Design review of the part built by this model. Coordinates are the model's own, in mm. Face numbers are marked on the shaded views. A direction names the side the tool comes from. Give positions to 0.01 mm unless a question says otherwise; leave off trailing zeros. Loops run counter-clockwise (first coordinate to the right, second up) from the corner with the lowest first, then second, coordinate; pieces in that order, holes last. Notation, with made-up numbers: (53.25, 43) -> (86.25, 43) arc R16 cw to (86.25, 62) -> close; hole circle Ø10 at (-10.5, 67). An arc over 180 degrees is marked (long way). Answer in a Markdown table with one row per item. Add a question column.
(1) Consider section D-D on y = 14.25. Write out the cut boundary in (x, z).
(2) For the marked faces 4 and 5, list the 3-axis set-ups (+Z, -Z, +X, -X, +Y, -Y) from which the entire face can be reached by the end or side of a thin tool; tool diameter is ignored.
(3) Draft analysis for pull direction X (two halves, no side actions). For the marked faces 1, 2 and 3, state which applies: +X half, -X half, draft (parallel to the pull), parting line (faces both ways), or undercut.
(4) Consider section B-B on x = 0. Write out the cut boundary in (y, z), then the cut area to 3 significant figures.
(5) Consider section C-C on y = 7. Write out the cut boundary in (x, z), then the cut area to 3 significant figures.
(6) Consider section A-A on z = 0. Write out the cut boundary in (x, y).
(7) For pin 1 (6 mm diameter, centred on x = -0.5, y = 9, fed in from +Z); pin 2 (3.5 mm diameter, centred on x = 0, z = 0, fed in from -Y); pin 3 (1.5 mm diameter, centred on y = 6, z = -4, fed in from -X); pin 4 (8 mm diameter, centred on x = 5, y = 15, fed in from +Z), all flat-tipped, find the tip position at first contact; note any pin that passes through.
(8) For line 1 (X direction, y = 18, z = 0); line 2 (X direction, y = 12.75, z = 0); line 3 (Z direction, x = -1.75, y = 16), list the stretches that pass through material, from the lowest coordinate up.
from build123d import *

# Parameters (mm, degrees)
FILLET_1_R = 3
FILLET_2_R = 1


with BuildPart() as part:
    # 草图1 → 旋转1 (revolve)
    with BuildSketch(Plane.XY, mode=Mode.PRIVATE) as revolve_1_sk:
        Polygon((3, 25), (3, 0), (6, 0), (6, 13), (9, 13), (9, 25), align=None)
    revolve(revolve_1_sk.sketch.rotate(Axis((0, 0, 0), (0, 1, 0)), 90), axis=Axis((0, 0, 0), (0, 1, 0)))

    # 圆角1
    fillet_1_edges = [part.edges().sort_by_distance(p)[0] for p in [
        (0, 25, 9),
    ]]
    fillet(fillet_1_edges, radius=FILLET_1_R)

    # 圆角2
    fillet_2_edges = [part.edges().sort_by_distance(p)[0] for p in [
        (0, 0, 6),
    ]]
    fillet(fillet_2_edges, radius=FILLET_2_R)


solid = part.part
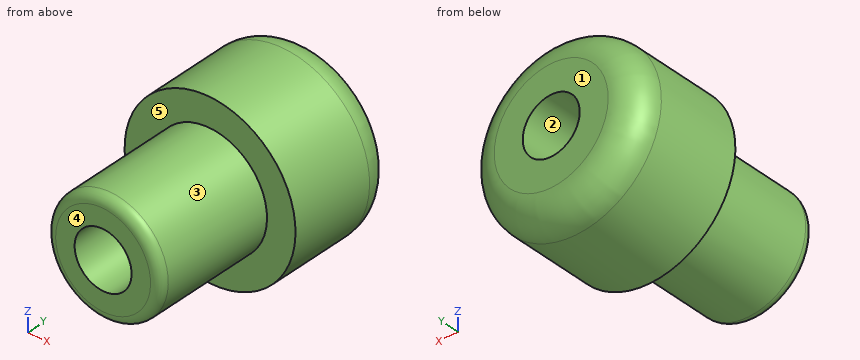
Values follow:
| question | item | result |
|---|---|---|
| 1 | outline | circle Ø18 at (0, 0); hole circle Ø6 at (0, 0) |
| 2 | face 4 | +Z, -Z, +X, -X, -Y |
| 2 | face 5 | -Y |
| 3 | face 1 | draft |
| 3 | face 2 | undercut |
| 3 | face 3 | parting line |
| 4 | outline | (0, -5) arc R1 ccw to (1, -6) -> (13, -6) -> (13, -9) -> (22, -9) arc R3 ccw to (25, -6) -> (25, -3) -> (0, -3) -> close; (0, 3) -> (25, 3) -> (25, 6) arc R3 ccw to (22, 9) -> (13, 9) -> (13, 6) -> (1, 6) arc R1 ccw to (0, 5) -> close |
| 4 | area | 218 mm2 |
| 5 | outline | circle Ø12 at (0, 0); hole circle Ø6 at (0, 0) |
| 5 | area | 84.8 mm2 |
| 6 | outline | (-9, 13) -> (-6, 13) -> (-6, 1) arc R1 ccw to (-5, 0) -> (-3, 0) -> (-3, 25) -> (-6, 25) arc R3 ccw to (-9, 22) -> close; (3, 0) -> (5, 0) arc R1 ccw to (6, 1) -> (6, 13) -> (9, 13) -> (9, 22) arc R3 ccw to (6, 25) -> (3, 25) -> close |
| 7 | pin 1 | z = 6 |
| 7 | pin 2 | through |
| 7 | pin 3 | x = -5.04 |
| 7 | pin 4 | z = 8.94 |
| 8 | line 1 | -9 to -3, 3 to 9 |
| 8 | line 2 | -6 to -3, 3 to 6 |
| 8 | line 3 | -8.83 to -2.44, 2.44 to 8.83 |
